Can you work these out from the drawing? Everything is in mm from the part's minimum corner. A direction names the side the tool comes from. Give positions to 0.01 mm unless a question says otherwise; leave off trailing zeros. Write each loop counter-clockwise with the first axis right and the second up, starting at its lowest first coordinate (ties: lowest second). Pieces come first, ordered by that corner, then holes. Notation, with made-up numbers: (73.25, 50.5) - (131.25, 50.5) arc R24 cw to (131.25, 66.5) - close; hole circle Ø7 at (-9.75, -7.5). An arc over 180 degrees is marked (long way). Write each question's results on one line, items separated by ' | '. Start each with the question number.
Item 1: Suppose I cut it at A-A on z = 118.5. List the corners of the cut face in (x, y) for me, then the cut area to 3 significant figures.
Item 2: Suppose I cut it at B-B on y = 339. List the corners of the cut face in (x, z) for me, then the cut area to 4 significant figures.
Item 3: Please list where these lines run through material, in increasing order: line 1 along X through (y, z) = (206, 640); line 2 along Y through (x, z) = (87, 119.5).
Item 4: Suppose I cut it at C-C on z = 427. List the corners of the cut face in (x, y) for me, then the cut area to 3 significant figures.
Item 5: Will these pins go through, and if not, where does the flat tip stop? P1, Ø1, axis at y = 63.5, z = 1560.5, coming from the -X side; P2, Ø4, axis at x = 117.5, z = 1547, coming from the +Y side.
Item 6: Which directions (+Z, -Z, +X, -X, +Y, -Y) give clear straight access to the entire face, cutting with the end or side of a thin tool? Please do the marked faces 1 and 2.
Item 7: Suppose I cut it at D-D on x = 271. List the corners of the cut face in (y, z) for me, then the cut area to 4 significant figures.
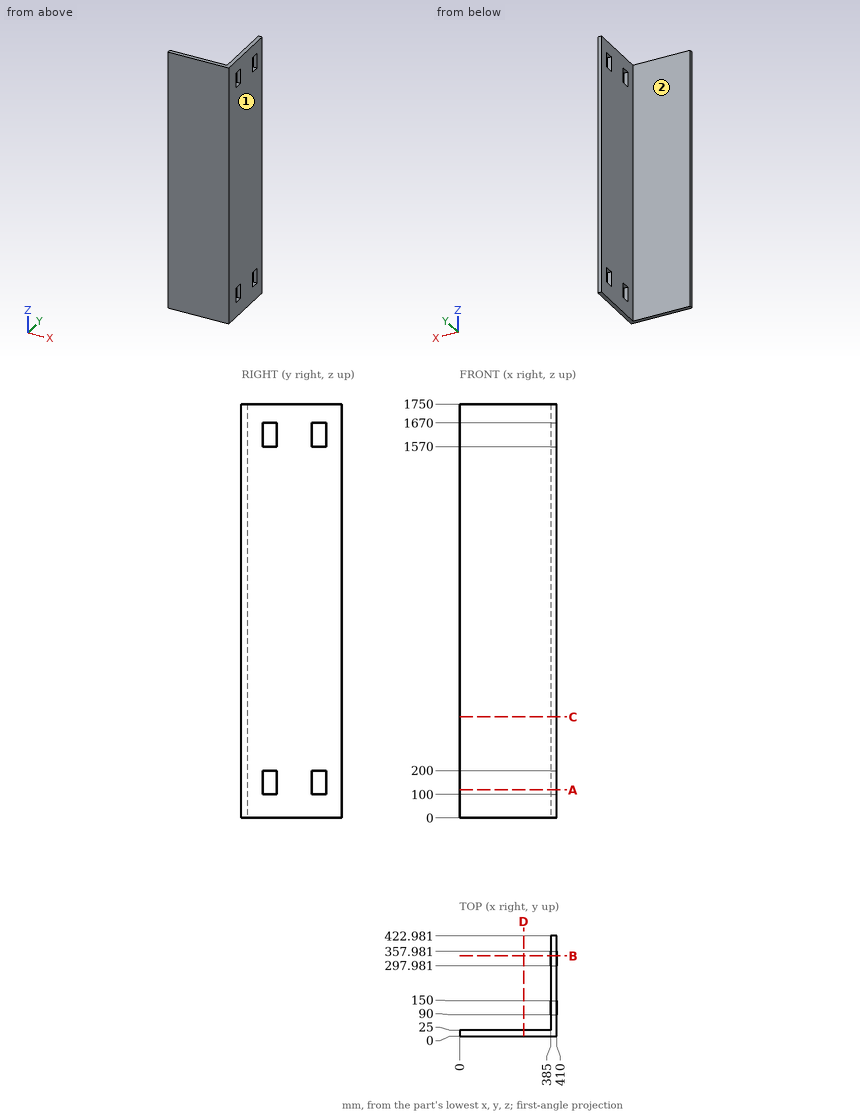
Checked values:
1) outline: (0, 0) - (410, 0) - (410, 90) - (385, 90) - (385, 25) - (0, 25) - close; (385, 150) - (410, 150) - (410, 297.98) - (385, 297.98) - close; (385, 357.98) - (410, 357.98) - (410, 422.98) - (385, 422.98) - close | area: 17,200 mm^2
2) outline: (385, 0) - (410, 0) - (410, 100) - (385, 100) - close; (385, 200) - (410, 200) - (410, 1570) - (385, 1570) - close; (385, 1670) - (410, 1670) - (410, 1750) - (385, 1750) - close | area: 38,750 mm^2
3) line 1: x = 385 to 410 | line 2: y = 0 to 25
4) outline: (0, 0) - (410, 0) - (410, 422.98) - (385, 422.98) - (385, 25) - (0, 25) - close | area: 20,200 mm^2
5) P1: stops at x = 385 | P2: stops at y = 25
6) face 1: +Z, -Z, +X, +Y, -Y | face 2: +Z, -Z, -X, +Y
7) outline: (0, 0) - (25, 0) - (25, 1750) - (0, 1750) - close | area: 43,750 mm^2
